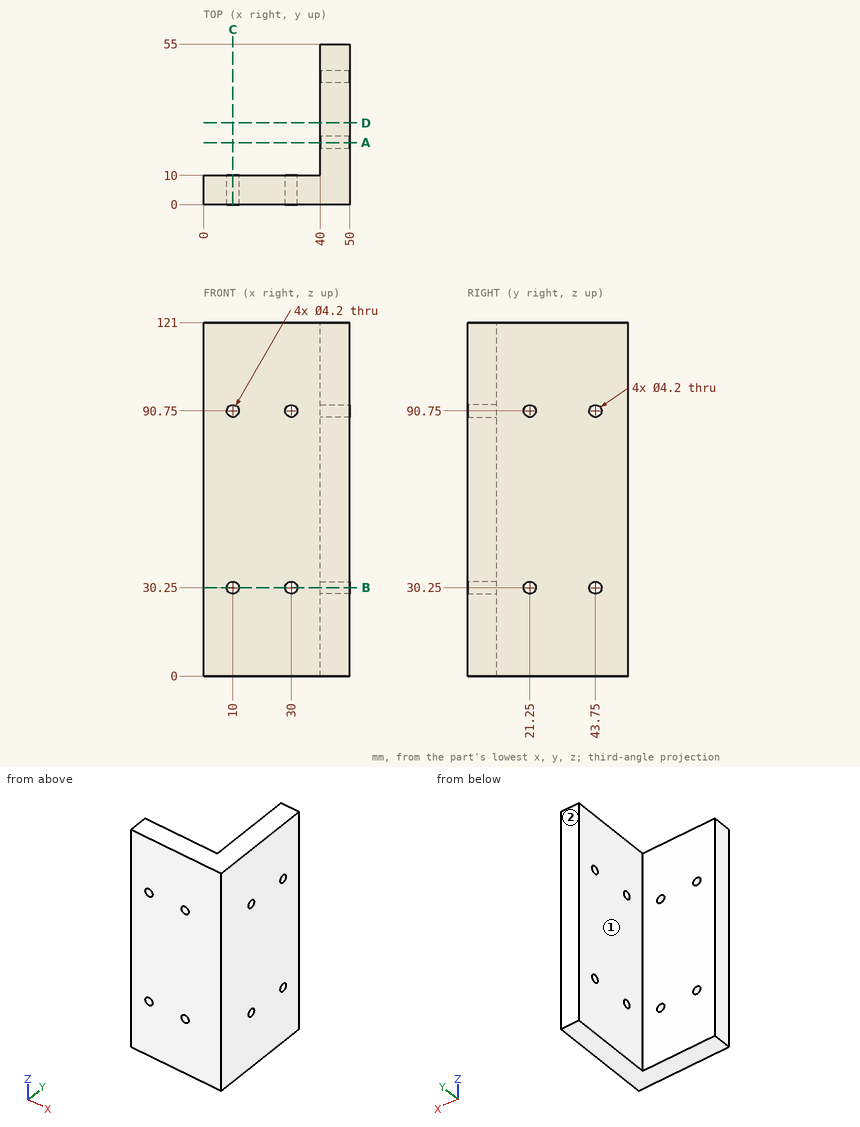
Verification items for this drawing (mm, ordinates from the low corner). A direction names the side the tool comes from. Round coordinates to 2 decimals unless told otherwise and drop trailing zeros. Order: outer loops, then holes, each group sorted by start corner. A loop starts at its lowest first (then second) coordinate and runs counter-clockwise, first axis right, second up. Notation, with made-up numbers: (78, 25) -> (116, 25) arc R21 ccw to (116, 41) -> close; hole circle Ø3 at (8, 53). An arc over 180 degrees is marked (long way). Use one line per item in the form item = value.
1. Scan lines: line 1 along X through (y, z) = (5.75, 90.75); line 2 along Y through (x, z) = (43, 30); line 3 along Y through (x, z) = (9, 109.5). Record each from-to range of solid material in increasing order. Write a range as from..to.
Working result:
line_1 = 0..7.9, 12.1..27.9, 32.1..50
line_2 = 0..19.16, 23.34..41.66, 45.84..55
line_3 = 0..10
2. Set-up check for the marked faces 1 and 2: record each of +Z, -Z, +X, -X, +Y, -Y from which the full face is reachable in a straight line by a thin tool's end or side.
Working result:
face_1 = +Z, -Z, -X, +Y
face_2 = +Z, -Z, +X, -X, +Y
3. Cross-section at C-C, the plane x = 10. Enter the section's corners in (y, z).
Working result:
outline = (0, 0) -> (10, 0) -> (10, 28.15) -> (0, 28.15) -> close; (0, 32.35) -> (10, 32.35) -> (10, 88.65) -> (0, 88.65) -> close; (0, 92.85) -> (10, 92.85) -> (10, 121) -> (0, 121) -> close
4. Cross-section at A-A, the plane y = 21.25. Enter the section's corners in (x, z).
Working result:
outline = (40, 0) -> (50, 0) -> (50, 28.15) -> (40, 28.15) -> close; (40, 32.35) -> (50, 32.35) -> (50, 88.65) -> (40, 88.65) -> close; (40, 92.85) -> (50, 92.85) -> (50, 121) -> (40, 121) -> close
5. Cross-section at B-B, the plane z = 30.25. Enter the section's corners in (x, y), plus the area to 3 significant figures.
Working result:
outline = (0, 0) -> (7.9, 0) -> (7.9, 10) -> (0, 10) -> close; (12.1, 0) -> (27.9, 0) -> (27.9, 10) -> (12.1, 10) -> close; (32.1, 0) -> (50, 0) -> (50, 19.15) -> (40, 19.15) -> (40, 10) -> (32.1, 10) -> close; (40, 23.35) -> (50, 23.35) -> (50, 41.65) -> (40, 41.65) -> close; (40, 45.85) -> (50, 45.85) -> (50, 55) -> (40, 55) -> close
area = 782 mm^2
6. Cross-section at D-D, the plane y = 28. Enter the section's corners in (x, z), plus the area to 3 significant figures.
Working result:
outline = (40, 0) -> (50, 0) -> (50, 121) -> (40, 121) -> close
area = 1,210 mm^2
7. Go/stop test with flat-tipped pins: pin 1 (22.5 mm diameter, centred on y = 42.5, z = 81, fed in from -X); pin 2 (5.5 mm diameter, centred on x = 30, z = 30.25, fed in from +Y). Record where each tip stops, or that it passes through.
Working result:
pin_1 = 40
pin_2 = 10
